Check sheet for the modelled part. Datum: model origin and axes. Units: mm. Face numbers are marked on the shaded views. A direction names the side the tool comes from. Give positions to 0.01 mm unless a question says otherwise; leave off trailing zeros. Order: outer loops, then holes, each group sorted by start corner. A loop starts at its lowest first (then second) coordinate and runs counter-clockwise, first axis right, second up.
from build123d import *

# Parameters (mm, degrees)
BASE_DISC_SKETCH_60_R       = 30
BASE_DISC_60_DEPTH          = 10
BASE_START                  = -10
BASE_PROFILE_CUT_DEPTH      = 10
COLLAR_SKETCH_40_R          = 20
COLLAR_40_DEPTH             = 40
SHAFT_SKETCH_26_R           = 13
SHAFT_26_DEPTH              = 60
SHAFT_END_FILLET_R3_R       = 3
SHAFT_FLAT_CUT_DEPTH        = 30
MOUNTING_FLANGE_SKETCH_74_W = 74
MOUNTING_FLANGE_SKETCH_74_H = 74
MOUNTING_FLANGE_74_DEPTH    = 10
MOUNTING_EAR_DEPTH          = 10
EAR_HOLE_SKETCH_10_R        = 5
EAR_HOLE_10_DEPTH           = 138.640836963


with BuildPart() as part:
    # Base Disc Sketch Ø60 → Base Disc Ø60 (new body)
    with BuildSketch(Plane.XY):
        Circle(BASE_DISC_SKETCH_60_R)
    extrude(amount=BASE_DISC_60_DEPTH)

    # Base Profile Cut Sketch → Base Profile Cut (cut)
    with BuildSketch(Plane.XY.offset(10).offset(BASE_START)):
        with BuildLine():
            Line((0, 18), (-24, 18))
            ThreePointArc((-24, 18), (0, 30), (24, 18))
            Line((24, 18), (0, 18))
        make_face()
        with BuildLine():
            Line((0, -18), (24, -18))
            ThreePointArc((24, -18), (0, -30), (-24, -18))
            Line((-24, -18), (0, -18))
        make_face()
    extrude(amount=BASE_PROFILE_CUT_DEPTH, mode=Mode.SUBTRACT)

    # Collar Sketch Ø40 → Collar Ø40 (add)
    with BuildSketch(Plane.XY.offset(10)):
        with Locations(Location((0, 0, 0), (0, 0, 115.841932763))):
            Circle(COLLAR_SKETCH_40_R)
    extrude(amount=COLLAR_40_DEPTH)

    # Shaft Sketch Ø26 → Shaft Ø26 (add)
    with BuildSketch(Plane.XY.offset(50)):
        Circle(SHAFT_SKETCH_26_R)
    extrude(amount=SHAFT_26_DEPTH)

    # Shaft End Fillet R3
    shaft_end_fillet_r3_edges = [part.edges().sort_by_distance(p)[0] for p in [
        (-13, 0, 110),
    ]]
    fillet(shaft_end_fillet_r3_edges, radius=SHAFT_END_FILLET_R3_R)

    # Shaft Flat Sketch → Shaft Flat Cut (cut)
    with BuildSketch(Plane(origin=(0, 0, 0), x_dir=(0, 0, -1), z_dir=(1, 0, 0))):
        Polygon((-107, 20.022291402), (-120.828706591, 20.022291402), (-120.828706591, -20.022291402), (-107, -20.022291402), (-50, -20.022291402), (-50, 20.022291402), align=None)
    extrude(amount=-SHAFT_FLAT_CUT_DEPTH, mode=Mode.SUBTRACT)

    # Mounting Flange Sketch 74 → Mounting Flange 74 (add)
    with BuildSketch(Plane(origin=(0, 0, 0), x_dir=(-1, 0, 0), z_dir=(0, 0, -1))):
        Rectangle(MOUNTING_FLANGE_SKETCH_74_W, MOUNTING_FLANGE_SKETCH_74_H)
    extrude(amount=MOUNTING_FLANGE_74_DEPTH)

    # Mounting Ear Sketch → Mounting Ear (add)
    with BuildSketch(Plane(origin=(37, 0, 0), x_dir=(0, 0, -1), z_dir=(1, 0, 0))):
        with BuildLine():
            Line((10, 37), (52.377859531, 13.060137394))
            ThreePointArc((52.377859531, 13.060137394), (60, 0), (52.377859531, -13.060137394))
            Line((52.377859531, -13.060137394), (10, -37))
            Line((10, -37), (10, 37))
        make_face()
    mounting_ear = extrude(amount=-MOUNTING_EAR_DEPTH)

    # Mounting Ear Mirror: Mounting Ear across plane
    add(mounting_ear.mirror(Plane(origin=(0, 0, 0), x_dir=(0, 0, 1), z_dir=(1, 0, 0))))

    # Ear Hole Sketch Ø10 → Ear Hole Ø10 (cut, through all)
    with BuildSketch(Plane(origin=(37, 0, 0), x_dir=(0, 0, -1), z_dir=(1, 0, 0))):
        with Locations((45, 0)):
            Circle(EAR_HOLE_SKETCH_10_R)
    extrude(amount=-EAR_HOLE_10_DEPTH, mode=Mode.SUBTRACT)


solid = part.part
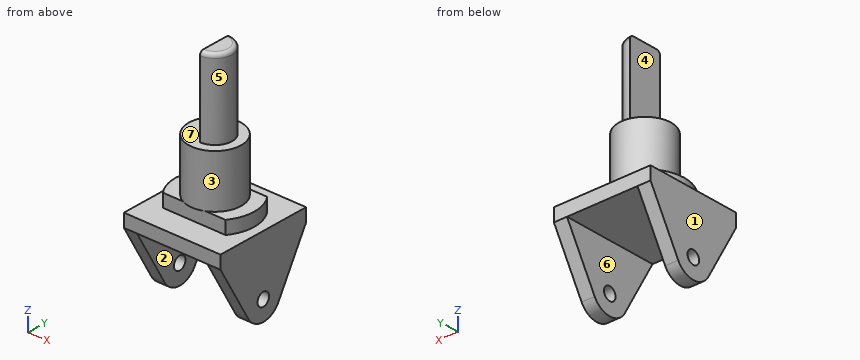
1) Section check C-C, the plane x = -17.5. Record the cut outline in (y, z), then the cut area to 3 significant figures.
Recorded:
outline: (-37, -10) - (37, -10) - (37, 0) - (18, 0) - (18, 10) - (9.68, 10) - (9.68, 50) - (-9.68, 50) - (-9.68, 10) - (-18, 10) - (-18, 0) - (-37, 0) - close
area: 1,870 mm2
2) Set-up check for the marked faces 1, 2, 3 and 4: record each of +Z, -Z, +X, -X, +Y, -Y from which the full face is reachable in a straight line by a thin tool's end or side.
Recorded:
face 1: +Z, -Z, -X, +Y, -Y
face 2: -Z, +Y, -Y
face 3: +Z
face 4: +Z, -X, +Y, -Y
3) Section check B-B, the plane z = -45. Record the cut outline in (x, y), then the cut area to 3 significant figures.
Recorded:
outline: (-37, -17.23) - (-27, -17.23) - (-27, -5) - (-37, -5) - close; (-37, 5) - (-27, 5) - (-27, 17.23) - (-37, 17.23) - close; (27, -17.23) - (37, -17.23) - (37, -5) - (27, -5) - close; (27, 5) - (37, 5) - (37, 17.23) - (27, 17.23) - close
area: 489 mm2
4) Section check D-D, the plane y = -22. Record the cut outline in (x, z).
Recorded:
outline: (-37, -36.55) - (-27, -36.55) - (-27, -10) - (27, -10) - (27, -36.55) - (37, -36.55) - (37, 0) - (-37, 0) - close
5) Material ranges on L1, parallel to Z at x = -26, y = 7; L2, parallel to Z at x = -3, y = 11.5; L3, parallel to Y at x = 32.5, z = -45, recorded low to high.
Recorded:
L1: z = -10 to 10
L2: z = -10 to 50
L3: y = -17.23 to -5, 5 to 17.23
6) Section check A-A, the plane y = 0. State how many separate pieces and enclosed holes the cut face has, then the cut area to 3 significant figures.
Recorded:
separate pieces: 3
enclosed holes: 0
area: 4,520 mm2
7) Draft check along X on the marked faces 5, 6 and 7. Enter one of: +X half, -X half, draft (parallel to the pull), parting line (faces both ways), or undercut.
Recorded:
face 5: +X half
face 6: undercut
face 7: draft
8) Depth check by flat-ended pin: pin 1 Ø1 at (x, y) = (-17, 6) entering from -Z; pin 2 Ø6.5 at (x, y) = (19.5, 4.5) entering from +Z; pin 3 Ø6 at (x, z) = (-3.5, 30.5) entering from +Y. Enter the tip coordinate at first touch or a pass-through.
Recorded:
pin 1: stops at z = -10
pin 2: stops at z = 50
pin 3: stops at y = 19.99
